Read the model definition and answer for the solid it produces. Units are mm, in the model's axes. A direction names the side the tool comes from. Coordinates: 2 decimals unless noted, no trailing zeros. Loops run counter-clockwise (first coordinate to the right, second up) from the corner with the lowest first, then second, coordinate; pieces in that order, holes last. Notation, with made-up numbers: M 23,12 L 51,12 A15 ccw 51,31 Z; hole C 6.5,62.5 d10. An arc over 180 degrees is marked long. Put each result on its own line as item: value.
from build123d import *

# Parameters (mm, degrees)
SKETCH1_R           = 15
SKETCH1_R_2         = 10
BOSS_EXTRUDE1_DEPTH = 15
SKETCH2_R           = 10
BOSS_EXTRUDE2_DEPTH = 5
CHAMFER1_SIZE       = 0.5


with BuildPart() as part:
    # Sketch1 → Boss-Extrude1 (new body)
    with BuildSketch(Plane.XY):
        Circle(SKETCH1_R)
        Circle(SKETCH1_R_2, mode=Mode.SUBTRACT)
    extrude(amount=BOSS_EXTRUDE1_DEPTH)

    # Sketch2 → Boss-Extrude2 (add)
    with BuildSketch(Plane.XY.offset(15)):
        with BuildLine():
            Line((-5.916079783, 17), (5.916079783, 17))
            ThreePointArc((5.916079783, 17), (18, 0), (5.916079783, -17))
            Line((5.916079783, -17), (-5.916079783, -17))
            ThreePointArc((-5.916079783, -17), (-18, 0), (-5.916079783, 17))
        make_face()
        Circle(SKETCH2_R, mode=Mode.SUBTRACT)
    extrude(amount=BOSS_EXTRUDE2_DEPTH)

    # Chamfer1
    chamfer1_edges = [part.edges().sort_by_distance(p)[0] for p in [
        (-10, 0, 20),
        (-10, 0, 0),
    ]]
    chamfer(chamfer1_edges, length=CHAMFER1_SIZE)


solid = part.part
1) Which of the six approach directions +Z, -Z, +X, -X, +Y, -Y give full straight-line access (tool end or side, diameter ignored) to faces 4 (the cylindrical face through (-14.985, 0.66, 7.395)), 5 (the flat face through (0, 17, 17))?
Answer list:
face 4: -Z
face 5: +Z, -Z, +X, -X, +Y
2) Find section A-A, the plane y = 0. Write down the section's boundary in (x, z).
Answer list:
outline: M -18,15 L -15,15 L -15,0 L -10.5,0 L -10,0.5 L -10,19.5 L -10.5,20 L -18,20 Z; M 10,0.5 L 10.5,0 L 15,0 L 15,15 L 18,15 L 18,20 L 10.5,20 L 10,19.5 Z
3) Straight lines are drawn through the part: line 1 (Y direction, x = 0, z = 14.75); line 2 (X direction, y = -1, z = 18.5); line 3 (Z direction, x = -2, y = 15). For each, find the intervals that lie inside material, in ascending order. Write a range as [from, to].
Answer list:
line 1: y = [-15, -10], [10, 15]
line 2: x = [-17.97, -9.95], [9.95, 17.97]
line 3: z = [15, 20]
4) Find section C-C, the plane z = 3.25. Write down the section's boundary in (x, y).
Answer list:
outline: C 0,0 d30; hole C 0,0 d20
5) Find section B-B, the plane x = 0. Write down the section's boundary in (y, z).
Answer list:
outline: M -17,15 L -15,15 L -15,0 L -10.5,0 L -10,0.5 L -10,19.5 L -10.5,20 L -17,20 Z; M 10,0.5 L 10.5,0 L 15,0 L 15,15 L 17,15 L 17,20 L 10.5,20 L 10,19.5 Z
6) Given pin 1 Ø4 at (x, z) = (11, 8) entering from -Y; pin 2 Ø4 at (x, z) = (14, 8.5) entering from +Y; pin 3 Ø1 at (y, z) = (11, 9) entering from -X, each flat-ended and moving along its own axis, determine where each tip first touches the part or whether it passes through.
Answer list:
pin 1: stops at y = -12
pin 2: stops at y = 9
pin 3: stops at x = -10.71
7) Determine the mould class of faces 1 (the cylindrical face through (-18, 0, 17)), 2 (the flat face through (-7.75, -7.32, 20)), 3 (the cylindrical face through (-2.17, -9.76, 9.87)) for opening direction X: released by +X, released by -X, zero draft, split by the parting line, or undercut.
Answer list:
face 1: released by -X
face 2: zero draft
face 3: undercut
8) Find section D-D, the plane y = -11.5. Write down the section's boundary in (x, z).
Answer list:
outline: M -13.85,15 L -9.63,15 L -9.63,0 L 9.63,0 L 9.63,15 L 13.85,15 L 13.85,20 L -13.85,20 Z
